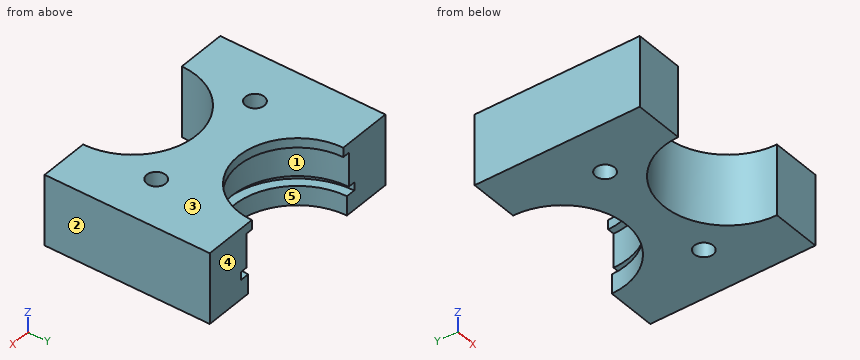
from build123d import *

# Parameters (mm, degrees)
SKETCH_1_W               = 480
SKETCH_1_H               = 350
EXTRUDE_1_DEPTH          = 150
CUT_EXTRUDE_1_DEPTH      = 333.753662639
CUT_EXTRUDE_1_DEPTH_BACK = 333.753662639
SKETCH_2_R               = 20
CUT_EXTRUDE_2_DEPTH      = 333.753662639
CUT_EXTRUDE_2_DEPTH_BACK = 333.753662639
SKETCH_3_R               = 135
SKETCH_3_R_2             = 125


with BuildPart() as part:
    # 草图1 → 凸台-拉伸1 (new body)
    with BuildSketch(Plane.XY):
        Rectangle(SKETCH_1_W, SKETCH_1_H)
    extrude(amount=EXTRUDE_1_DEPTH)

    # 草图2 → 切除-拉伸1 (cut, two sides: drawn at the far end of the back side and taken through both)
    with BuildSketch(Plane.XY.offset(150).offset(-CUT_EXTRUDE_1_DEPTH_BACK)):
        with Locations((-135, -20)):
            Circle(SKETCH_2_R)
        with Locations((135, -20)):
            Circle(SKETCH_2_R)
    extrude(amount=CUT_EXTRUDE_1_DEPTH + CUT_EXTRUDE_1_DEPTH_BACK, mode=Mode.SUBTRACT)

    # 草图3 → 切除-拉伸2 (cut, two sides: drawn at the far end of the back side and taken through both)
    with BuildSketch(Plane.XY.offset(150).offset(-CUT_EXTRUDE_2_DEPTH_BACK)):
        with Locations((0, -175)):
            Circle(SKETCH_3_R)
        with Locations((0, 175)):
            Circle(SKETCH_3_R_2)
    extrude(amount=CUT_EXTRUDE_2_DEPTH + CUT_EXTRUDE_2_DEPTH_BACK, mode=Mode.SUBTRACT)

    # 草图5 → 切除-旋转1 (revolve, cut)
    with BuildSketch(Plane(origin=(0, 175, 0), x_dir=(1, 0, 0), z_dir=(0, 1, 0))):
        Polygon((0, -130), (-140, -130), (-140, -58), (-155, -58), (-155, -41), (-135, -41), (-135, 0), (0, 0), (0, -41), align=None)
    revolve(axis=Axis((0, 175, 150), (0, 0, -1)), mode=Mode.SUBTRACT)


solid = part.part
Read the model definition and answer for the solid it produces. Units are mm, in the model's axes. Face numbers are marked on the shaded views. A direction names the side the tool comes from. Give positions to 0.01 mm unless a question says otherwise; leave off trailing zeros. Write each loop counter-clockwise with the first axis right and the second up, starting at its lowest first coordinate (ties: lowest second). Pieces come first, ordered by that corner, then holes. Notation, with made-up numbers: M 12.25,36.5 L 24.25,36.5 A14 ccw 24.25,51.5 Z; hole C 4,38.5 d1. An arc over 180 degrees is marked long. One line per item, written item: value. Start each with the question number.
(1) A tool of negligible diameter and unlimited length cuts with its end or side. For the marked faces 4 and 5, from which of +Z, -Z, +X, -X, +Y, -Y can it reach the whole face along a straight path? Write none if from no direction.
(2) Determine the mould class of the marked faces 1, 2 and 3 for opening direction X: pulls with the +X half, pulls with the -X half, needs draft (parallel to the pull), parting line crosses it, or undercut.
(3) Find the intervals of material crossed by line 1 (X direction, y = -20, z = 30.5); line 2 (X direction, y = -24.5, z = 72); line 3 (X direction, y = 74.5, z = 88.5), in increasing order.
(4) A flat-ended cylindrical pin translates along its axis: pin 1 Ø10 at (x, z) = (28.5, 114.5) entering from +Y. Find the tip coordinate at first contact, or state that the pin passes through.
(5) Find section D-D (y = -20). Determine the outline of the cut face in (x, z).
(6) Find section B-B (y = 60.5). Determine the outline of the cut face in (x, z).
(7) Find section C-C (x = 145.5). Determine the outline of the cut face in (y, z), plus the area to 3 significant figures.
(8) Find section A-A (z = 32). Determine the outline of the cut face in (x, y), plus the area to 3 significant figures.
Results below:
1. face 4: +Z, -Z, +X, -X, +Y
1. face 5: -Z, +Y
2. face 1: undercut
2. face 2: pulls with the +X half
2. face 3: needs draft
3. line 1: x = -240 to -155, -115 to 115, 155 to 240
3. line 2: x = -240 to -154.49, -115.51 to 115.51, 154.49 to 240
3. line 3: x = -240 to -97.47, 97.47 to 240
4. pin 1: stops at y = 39.07
5. outline: M -240,0 L -155,0 L -155,150 L -240,150 Z; M -115,0 L 115,0 L 115,150 L -115,150 Z; M 155,0 L 240,0 L 240,150 L 155,150 Z
6. outline: M -240,0 L -71.52,0 L -71.52,41 L -104.47,41 L -104.47,58 L -80.56,58 L -80.56,130 L -50.15,130 L -50.15,150 L -240,150 Z; M 50.15,130 L 80.56,130 L 80.56,58 L 104.47,58 L 104.47,41 L 71.52,41 L 71.52,0 L 240,0 L 240,150 L 50.15,150 Z
7. outline: M -175,0 L -37.02,0 L -37.02,150 L -175,150 Z; M -2.98,0 L 175,0 L 175,41 L 121.57,41 L 121.57,58 L 175,58 L 175,150 L -2.98,150 Z
7. area: 46,500 mm^2
8. outline: M -240,-175 L -135,-175 A135 cw 135,-175 L 240,-175 L 240,175 L 135,175 A135 cw -135,175 L -240,175 Z; hole C -135,-20 d40; hole C 135,-20 d40
8. area: 108,000 mm^2
